```python
from build123d import *

# Parameters (mm, degrees)
BOSS_EXTRUDE2_DEPTH = 17.5
SKETCH3_R           = 5.5
CUT_EXTRUDE2_DEPTH  = 54
SKETCH4_R           = 11
BOSS_EXTRUDE3_DEPTH = 260
SKETCH5_R           = 7.5
BOSS_EXTRUDE4_DEPTH = 55
SKETCH6_R           = 6
BOSS_EXTRUDE5_DEPTH = 20
CHAMFER1_SIZE       = 1


with BuildPart() as part:
    # Sketch1 → Boss-Extrude2 (new, symmetric)
    with BuildSketch(Plane.XY):
        with BuildLine():
            Line((-15, 20), (16.011299973, 20))
            ThreePointArc((16.011299973, 20), (18.83173681, 18.83173681), (20, 16.011299973))
            Line((20, 16.011299973), (20, -16.011299973))
            ThreePointArc((20, -16.011299973), (18.83173681, -18.83173681), (16.011299973, -20))
            Line((16.011299973, -20), (-16.011299973, -20))
            ThreePointArc((-16.011299973, -20), (-18.83173681, -18.83173681), (-20, -16.011299973))
            Line((-20, -16.011299973), (-20, 15))
            ThreePointArc((-20, 15), (-18.535533906, 18.535533906), (-15, 20))
        make_face()
    extrude(amount=BOSS_EXTRUDE2_DEPTH, both=True)

    # Sketch3 → Cut-Extrude2 (cut)
    with BuildSketch(Plane(origin=(0, 20, 0), x_dir=(1, 0, 0), z_dir=(0, 1, 0))):
        with Locations(Location((0, 0, 0), (0, 0, 270))):
            Circle(SKETCH3_R)
    extrude(amount=-CUT_EXTRUDE2_DEPTH, mode=Mode.SUBTRACT)

    # Sketch4 → Boss-Extrude3 (add)
    with BuildSketch(Plane(origin=(0, 0, -17.5), x_dir=(-1, 0, 0), z_dir=(0, 0, -1))):
        Circle(SKETCH4_R)
    extrude(amount=BOSS_EXTRUDE3_DEPTH)

    # Sketch5 → Boss-Extrude4 (add)
    with BuildSketch(Plane(origin=(0, 0, -277.5), x_dir=(-1, 0, 0), z_dir=(0, 0, -1))):
        Circle(SKETCH5_R)
    extrude(amount=BOSS_EXTRUDE4_DEPTH)

    # Sketch6 → Boss-Extrude5 (add)
    with BuildSketch(Plane(origin=(0, 0, -332.5), x_dir=(-1, 0, 0), z_dir=(0, 0, -1))):
        Circle(SKETCH6_R)
    extrude(amount=BOSS_EXTRUDE5_DEPTH)

    # Chamfer1
    chamfer1_edges = [part.edges().sort_by_distance(p)[0] for p in [
        (6, 0, -352.5),
    ]]
    chamfer(chamfer1_edges, length=CHAMFER1_SIZE)


solid = part.part
```
Could you check a few things on this model? Use its own coordinates, in mm. A direction names the side the tool comes from. Round coordinates to 2 decimals unless told otherwise and drop trailing zeros. Loops run counter-clockwise (first coordinate to the right, second up) from the corner with the lowest first, then second, coordinate; pieces in that order, holes last. Notation, with made-up numbers: M -12.75,70.5 L 11.25,70.5 A16 cw 11.25,97.5 Z; hole C 78.25,-3 d1. An arc over 180 degrees is marked long. Write item = value, one per line.
1. I want a section at A-A, the plane z = 0. Write out the boundary of the cut face in (x, y), and give its area (3 significant figures).
Results below:
outline = M -20,-16.01 A3.99 ccw -16.01,-20 L -5.5,-20 L -5.5,20 L -15,20 A5 ccw -20,15 Z; M 5.5,-20 L 16.01,-20 A3.99 ccw 20,-16.01 L 20,16.01 A3.99 ccw 16.01,20 L 5.5,20 Z
area = 1,140 mm²
2. Thinking about a two-plate mould opening in X: for faces 3 (the face through (-20, -1, 0)), 4 (the face through (-5.37, 0.28, -1.19)), 5 (the face through (-7.2, 2.6, -277.5)), 6 (the face through (6, 0, -342)), which applies, +X half, -X half, draft (parallel to the pull), parting line (faces both ways), or undercut?
Results below:
face_3 = -X half
face_4 = undercut
face_5 = draft
face_6 = parting line
3. I want a section at D-D, the plane z = -95. Write out the boundary of the cut face in (x, y), and give its area (3 significant figures).
Results below:
outline = C 0,0 d22
area = 380 mm²
4. I need wall thicknesses on probe 1 along X at (y, z) = (4, 0); probe 2 along Z at (x, y) = (14.5, 10); probe 3 along X at (y, z) = (-9.5, -73). Which ranges of each line are inside material? Lowest first, please.
Results below:
probe_1 = -20 to -5.5, 5.5 to 20
probe_2 = -17.5 to 17.5
probe_3 = -5.55 to 5.55
5. I want a section at C-C, the plane y = 0. Write out the boundary of the cut face in (x, z).
Results below:
outline = M -20,-17.5 L -11,-17.5 L -11,-277.5 L -7.5,-277.5 L -7.5,-332.5 L -6,-332.5 L -6,-351.5 L -5,-352.5 L 5,-352.5 L 6,-351.5 L 6,-332.5 L 7.5,-332.5 L 7.5,-277.5 L 11,-277.5 L 11,-17.5 L 20,-17.5 L 20,17.5 L -20,17.5 Z; hole C 0,0 d11
6. Which directions (+Z, -Z, +X, -X, +Y, -Y) give clear straight access to the entire face, cutting with the end or side of a thin tool? Please do faces 1 (the face through (2.38, -10.74, -145.68)), 2 (the face through (0, 0, -352.5)).
Results below:
face_1 = -Z
face_2 = -Z, +X, -X, +Y, -Y
7. I want a section at B-B, the plane x = 0. Write out the boundary of the cut face in (y, z).
Results below:
outline = M -20,-17.5 L -11,-17.5 L -11,-277.5 L -7.5,-277.5 L -7.5,-332.5 L -6,-332.5 L -6,-351.5 L -5,-352.5 L 5,-352.5 L 6,-351.5 L 6,-332.5 L 7.5,-332.5 L 7.5,-277.5 L 11,-277.5 L 11,-17.5 L 20,-17.5 L 20,-5.5 L -20,-5.5 Z; M -20,5.5 L 20,5.5 L 20,17.5 L -20,17.5 Z
8. Will these pins go through, and if not, where does the flat tip stop? P1, Ø3, axis at x = 11.5, z = -29, coming from the +Y side; P2, Ø5, axis at x = 6, z = -103.5, coming from the +Y side; P3, Ø2, axis at y = 8.5, z = -266.5, coming from the -X side.
Results below:
P1 = 4.58
P2 = 10.43
P3 = -8.05
